```python
from build123d import *

# Parameters (mm, degrees)
BOSS_EXTRUDE1_DEPTH = 8
SKETCH2_R           = 12.5
BOSS_EXTRUDE2_DEPTH = 40
LPATTERN1_COUNT     = 2
LPATTERN1_PITCH     = 48
SKETCH3_R           = 7.5
BOSS_EXTRUDE3_DEPTH = 12
LPATTERN2_COUNT     = 2
LPATTERN2_PITCH     = 68


with BuildPart() as part:
    # Sketch1 → Boss-Extrude1 (new body)
    with BuildSketch(Plane(origin=(0, 0, 0), x_dir=(1, 0, 0), z_dir=(0, 1, 0))):
        with BuildLine():
            ThreePointArc((0, 20), (-20, 0), (0, -20))
            ThreePointArc((0, -20), (30, -16.969384567), (60, -20))
            ThreePointArc((60, -20), (80, 0), (60, 20))
            ThreePointArc((60, 20), (30, 16.969384567), (0, 20))
        make_face()
    boss_extrude1 = extrude(amount=BOSS_EXTRUDE1_DEPTH)

    # Sketch2 → Boss-Extrude2 (add)
    with BuildSketch(Plane(origin=(0, 8, 0), x_dir=(1, 0, 0), z_dir=(0, 1, 0))):
        with Locations(Location((0, 0, 0), (0, 0, 270))):
            Circle(SKETCH2_R)
        with Locations(Location((60, 0, 0), (0, 0, 270))):
            Circle(SKETCH2_R)
    extrude(amount=BOSS_EXTRUDE2_DEPTH)

    # LPattern1: Boss-Extrude1 ×2
    with Locations(*[(0, i * LPATTERN1_PITCH, 0) for i in range(1, LPATTERN1_COUNT)]):
        add(boss_extrude1)

    # Sketch3 → Boss-Extrude3 (add)
    with BuildSketch(Plane(origin=(0, 56, 0), x_dir=(1, 0, 0), z_dir=(0, 1, 0))):
        with Locations(Location((0, 0, 0), (0, 0, 270))):
            Circle(SKETCH3_R)
        with Locations(Location((60, 0, 0), (0, 0, 270))):
            Circle(SKETCH3_R)
    boss_extrude3 = extrude(amount=BOSS_EXTRUDE3_DEPTH)

    # LPattern2: Boss-Extrude3 ×2
    with Locations(*[(0, -i * LPATTERN2_PITCH, 0) for i in range(1, LPATTERN2_COUNT)]):
        add(boss_extrude3)


solid = part.part
```
Geometry check sheet. Reference: the model listing, model coordinates, mm. A direction names the side the tool comes from. Give positions to 0.01 mm unless a question says otherwise; leave off trailing zeros. Order: outer loops, then holes, each group sorted by start corner. A loop starts at its lowest first (then second) coordinate and runs counter-clockwise, first axis right, second up. Notation, with made-up numbers: (16, 26) -> (26, 26) arc R16 cw to (26, 56) -> close; hole circle Ø1 at (73, 33.5). An arc over 180 degrees is marked (long way). Write each question's results on one line, items separated by ' | '. Start each with the question number.
(1) Gauge pin test, flat ends, axial feed: P1, Ø4, axis at y = 7, z = 4, coming from the +X side; P2, Ø12, axis at x = 20, z = -7.5, coming from the +Y side; P3, Ø3, axis at x = 2.5, y = 34.5, coming from the -Z side. Record the tip position at first contact, or that the pin passes through.
(2) Access from +Z, -Z, +X, -X, +Y, -Y to the whole of each face (thin tool, end or side, straight path). Record for faces 1 (the face through (67.436, 61.916, -0.976)), 2 (the face through (30.42, 51.94, -16.97)), 3 (the face through (29, 8, 0)), 4 (the face through (67.436, -6.084, -0.976)).
(3) Scan lines: line 1 (Y direction, x = 56.5, z = 18); line 2 (Y direction, x = 48.5, z = 4); line 3 (X direction, y = 35, z = -10). Record each from-to range of solid material in increasing order.
(4) Sectioned sample at D-D (x = 49). Enter the section's corners in (y, z).
(5) Mould release check, pull along Y, two halves, no side actions. Record for faces 5 (the face through (29, 56, 0)), 6 (the face through (72.394, 27.72, -1.627)), 7 (the face through (0.33, 61.916, -7.493)): pulls with the +Y half, pulls with the -Y half, needs draft (parallel to the pull), parting line crosses it, or undercut.
(6) Sectioned sample at B-B (y = 26). Enter the section's corners in (x, z).
(7) Sectioned sample at C-C (x = 14). Enter the section's corners in (y, z).
Answer below:
1) P1: x = 79.9 | P2: y = 56 | P3: z = -12.46
2) face 1: +Y | face 2: -Z, +Y, -Y | face 3: none | face 4: -Y
3) line 1: 0 to 8, 48 to 56 | line 2: 0 to 56 | line 3: -7.5 to 7.5, 52.5 to 67.5
4) outline: (0, -18.18) -> (8, -18.18) -> (8, -5.94) -> (48, -5.94) -> (48, -18.18) -> (56, -18.18) -> (56, 18.18) -> (48, 18.18) -> (48, 5.94) -> (8, 5.94) -> (8, 18.18) -> (0, 18.18) -> close
5) face 5: pulls with the +Y half | face 6: undercut | face 7: needs draft
6) outline: circle Ø25 at (0, 0); circle Ø25 at (60, 0)
7) outline: (0, -17.83) -> (8, -17.83) -> (8, 17.83) -> (0, 17.83) -> close; (48, -17.83) -> (56, -17.83) -> (56, 17.83) -> (48, 17.83) -> close
